from build123d import *

# Parameters (mm, degrees)
SKETCH1_R           = 3
BOSS_EXTRUDE1_DEPTH = 6


with BuildPart() as part:
    # Sketch1 → Boss-Extrude1 (new body)
    with BuildSketch(Plane.XY):
        with BuildLine():
            Line((0, 7.5), (140, 7.5))
            ThreePointArc((140, 7.5), (147.5, 0), (140, -7.5))
            Line((140, -7.5), (0, -7.5))
            ThreePointArc((0, -7.5), (-7.5, 0), (0, 7.5))
        make_face()
        Circle(SKETCH1_R, mode=Mode.SUBTRACT)
        with Locations((40, 0)):
            Circle(SKETCH1_R, mode=Mode.SUBTRACT)
        with Locations((140, 0)):
            Circle(SKETCH1_R, mode=Mode.SUBTRACT)
    extrude(amount=BOSS_EXTRUDE1_DEPTH)


solid = part.part
Input: part model. Units: mm. Frame: model coordinates. Round coordinates to 2 decimals unless told otherwise and drop trailing zeros. Write each loop counter-clockwise with the first axis right and the second up, starting at its lowest first coordinate (ties: lowest second). Pieces come first, ordered by that corner, then holes.
1) Cut plane D-D (y = 6). Return the cut outline in (x, z).
2) Contact query for a flat-ended pin moving along its axis: P1, Ø2, axis at y = 1.5, z = 0.5, coming from the +X side. Output: stop coordinate, or through.
3) Cut plane B-B (x = 40). Return the cut outline in (y, z), then the cut area to 3 significant figures.
4) Draft query along X for faces 1 (the cylindrical face through (-7.5, -0.16, 2.96)), 2 (the flat face through (71, 0, 6)), 3 (the cylindrical face through (147.5, 0.16, 2.96)), 4 (the cylindrical face through (142.86, 0.9, 2.96)). Return one class per face: pulls with the +X half, pulls with the -X half, needs draft (parallel to the pull), parting line crosses it, or undercut.
5) Cut plane C-C (z = 3.2). Return the cut outline in (x, y), then the cut area to 3 significant figures.
6) Ray query, L1, parallel to Y at x = 40, z = 4.4; L2, parallel to X at y = 1.75, z = 3.4; L3, parallel to X at y = 0.5, z = 1.55. Return the intervals inside material, ascending.
7) Cut plane A-A (y = 0). Return the cut outline in (x, z), then the cut area to 3 significant figures.
Geometry says:
1. outline: (-4.5, 0) - (144.5, 0) - (144.5, 6) - (-4.5, 6) - close
2. P1: stops at x = 147.48
3. outline: (-7.5, 0) - (-3, 0) - (-3, 6) - (-7.5, 6) - close; (3, 0) - (7.5, 0) - (7.5, 6) - (3, 6) - close
3. area: 54.0 mm2
4. face 1: pulls with the -X half
4. face 2: needs draft
4. face 3: pulls with the +X half
4. face 4: undercut
5. outline: (0, -7.5) - (140, -7.5) arc R7.5 ccw to (140, 7.5) - (0, 7.5) arc R7.5 ccw to start; hole circle Ø6 at (0, 0); hole circle Ø6 at (40, 0); hole circle Ø6 at (140, 0)
5. area: 2,190 mm2
6. L1: y = -7.5 to -3, 3 to 7.5
6. L2: x = -7.29 to -2.44, 2.44 to 37.56, 42.44 to 137.56, 142.44 to 147.29
6. L3: x = -7.48 to -2.96, 2.96 to 37.04, 42.96 to 137.04, 142.96 to 147.48
7. outline: (-7.5, 0) - (-3, 0) - (-3, 6) - (-7.5, 6) - close; (3, 0) - (37, 0) - (37, 6) - (3, 6) - close; (43, 0) - (137, 0) - (137, 6) - (43, 6) - close; (143, 0) - (147.5, 0) - (147.5, 6) - (143, 6) - close
7. area: 822 mm2
